Build history of the part. All positions in model axes, mm. A direction names the side the tool comes from. Round coordinates to 2 decimals unless told otherwise and drop trailing zeros. Write each loop counter-clockwise with the first axis right and the second up, starting at its lowest first coordinate (ties: lowest second). Pieces come first, ordered by that corner, then holes. Notation, with made-up numbers: M 39,36.25 L 56,36.25 A23 ccw 56,68.25 Z; hole C 40.25,6.5 d10. An arc over 180 degrees is marked long. Write item = value, one per line. Start each with the question number.
Q1. Tool access for faces 1 (the cylindrical face through (6.466, -2.681, 433.632)), 2 (the flat face through (2, 6, -376.8)): list every direction of +Z, -Z, +X, -X, +Y, -Y with a clear straight run to the whole face (end or side of a thin tool).
Q2. Band-saw the part on A-A on z = -255. Write the cut outline in (x, y).
Q3. Probe L1, parallel to Y at x = 0, z = -391.5; L2, parallel to X at y = 0, z = -393.25; L3, parallel to Z at x = 0.75, y = -7. List the from-to ranges inside material, lowest first.
Q4. Drop flat-ended pins along their axis: P1, Ø2, axis at y = 6.5, z = -155.5, coming from the -X side; P2, Ø1.5, axis at x = 3.5, y = -6, coming from the -Z side; P3, Ø1.1, axis at y = 5, z = -387, coming from the -X side. Give the stop position or say it passes through.
```python
from build123d import *

# Parameters (mm, degrees)
SKETCH_1_R               = 7
EXTRUDE_1_DEPTH          = 450
SKETCH_2_R               = 8.5
EXTRUDE_2_DEPTH          = 416.8
CUT_EXTRUDE_START        = -33.2
SKETCH_3_R               = 8.5
SKETCH_3_R_2             = 6
CUT_EXTRUDE_1_DEPTH      = 33.2
CUT_EXTRUDE_2_DEPTH      = 451.160526923
CUT_EXTRUDE_2_DEPTH_BACK = 451.160526923
SKETCH_4_W               = 12
SKETCH_4_H               = 12.45
MOVE_FACE_1_BY           = 40
MOVE_FACE_1_2_BY         = 40
CUT_EXTRUDE_11_DEPTH     = 2.5
HOLE_WIZARD_M4_1_D       = 3.3
HOLE_WIZARD_M4_1_DEPTH   = 10.1
HOLE_WIZARD_M4_1_TIP     = 0.991420021
CUT_EXTRUDE_START_2      = 1.1
SKETCH_35_R              = 8.5
SKETCH_35_R_2            = 8.1
CUT_EXTRUDE_12_DEPTH     = 1.1
SKETCH_36_R              = 8.5
SKETCH_36_R_2            = 8.1
CUT_EXTRUDE_13_DEPTH     = 1.1
SKETCH_37_R              = 8.5
SKETCH_37_R_2            = 8.1
CUT_EXTRUDE_14_DEPTH     = 1.1
SKETCH_38_R              = 8.5
SKETCH_38_R_2            = 8.1
CUT_EXTRUDE_15_DEPTH     = 1.1


with BuildPart() as part:
    # 草图1 → 凸台-拉伸1 (new, symmetric)
    with BuildSketch(Plane.XY):
        Circle(SKETCH_1_R)
    extrude(amount=EXTRUDE_1_DEPTH, both=True)

    # 草图2 → 凸台-拉伸2 (add, symmetric)
    with BuildSketch(Plane.XY):
        Circle(SKETCH_2_R)
    extrude(amount=EXTRUDE_2_DEPTH, both=True)

    # 草图3 → 切除-拉伸1 (cut)
    with BuildSketch(Plane(origin=(0, 0, -450), x_dir=(-1, 0, 0), z_dir=(0, 0, -1)).offset(CUT_EXTRUDE_START)):
        with Locations(Location((0, 0, 0), (0, 0, 180))):
            Circle(SKETCH_3_R)
        Circle(SKETCH_3_R_2, mode=Mode.SUBTRACT)
    extrude(amount=CUT_EXTRUDE_1_DEPTH, mode=Mode.SUBTRACT)

    # 草图4 → 切除-拉伸2 (cut, two sides: drawn at the far end of the back side and taken through both)
    with BuildSketch(Plane(origin=(0, 0, 0), x_dir=(1, 0, 0), z_dir=(0, 1, 0)).offset(-CUT_EXTRUDE_2_DEPTH_BACK)):
        with Locations((0, 443.775)):
            Rectangle(SKETCH_4_W, SKETCH_4_H)
    extrude(amount=CUT_EXTRUDE_2_DEPTH + CUT_EXTRUDE_2_DEPTH_BACK, mode=Mode.SUBTRACT)

    # Move Face 1: a face moved inward by 40.0
    extrude(part.faces().sort_by_distance((0, 0, -437.55))[0], amount=MOVE_FACE_1_BY, dir=(0, 0, 1), mode=Mode.SUBTRACT)

    # Move Face 1 2: a face moved inward by 40.0
    extrude(part.faces().sort_by_distance((0, -6.8, -416.8))[0], amount=MOVE_FACE_1_2_BY, dir=(0, 0, 1), mode=Mode.SUBTRACT)

    # 草图31 → 切除-拉伸11 (cut)
    with BuildSketch(Plane(origin=(0, 6, -397.55), x_dir=(0, 0, 1), z_dir=(0, 1, 0))):
        with BuildLine():
            Line((-1, 2), (17.75, 2))
            ThreePointArc((17.75, 2), (19.75, 0), (17.75, -2))
            Line((17.75, -2), (-1, -2))
            ThreePointArc((-1, -2), (-3, 0), (-1, 2))
        make_face()
    extrude(amount=-CUT_EXTRUDE_11_DEPTH, mode=Mode.SUBTRACT)

    # M4 螺纹孔1
    with Locations(Plane(origin=(0, 0, -397.55), x_dir=(-1, 0, 0), z_dir=(0, 0, -1))):
        with Locations((0, 0)):
            Hole(HOLE_WIZARD_M4_1_D / 2, depth=HOLE_WIZARD_M4_1_DEPTH)
            with Locations((0, 0, -(HOLE_WIZARD_M4_1_DEPTH + HOLE_WIZARD_M4_1_TIP / 2))):  # 118° drill point
                Cone(0, HOLE_WIZARD_M4_1_D / 2, HOLE_WIZARD_M4_1_TIP, mode=Mode.SUBTRACT)

    # 草图35 → 切除-拉伸12 (cut)
    with BuildSketch(Plane.XY.offset(319.2).offset(CUT_EXTRUDE_START_2)):
        Circle(SKETCH_35_R)
        Circle(SKETCH_35_R_2, mode=Mode.SUBTRACT)
    extrude(amount=-CUT_EXTRUDE_12_DEPTH, mode=Mode.SUBTRACT)

    # 草图36 → 切除-拉伸13 (cut)
    with BuildSketch(Plane.XY.offset(298.1).offset(CUT_EXTRUDE_START_2)):
        Circle(SKETCH_36_R)
        Circle(SKETCH_36_R_2, mode=Mode.SUBTRACT)
    extrude(amount=-CUT_EXTRUDE_13_DEPTH, mode=Mode.SUBTRACT)

    # 草图37 → 切除-拉伸14 (cut)
    with BuildSketch(Plane.XY.offset(-325.8).offset(CUT_EXTRUDE_START_2)):
        Circle(SKETCH_37_R)
        Circle(SKETCH_37_R_2, mode=Mode.SUBTRACT)
    extrude(amount=-CUT_EXTRUDE_14_DEPTH, mode=Mode.SUBTRACT)

    # 草图38 → 切除-拉伸15 (cut)
    with BuildSketch(Plane.XY.offset(-346.9).offset(CUT_EXTRUDE_START_2)):
        Circle(SKETCH_38_R)
        Circle(SKETCH_38_R_2, mode=Mode.SUBTRACT)
    extrude(amount=-CUT_EXTRUDE_15_DEPTH, mode=Mode.SUBTRACT)


solid = part.part
```
Conclusion:
q1.face_1 = +Z
q1.face_2 = -Z
q2.outline = C 0,0 d17
q3.L1 = -6 to -1.65, 1.65 to 3.5
q3.L2 = -6 to -1.65, 1.65 to 6
q3.L3 = -376.8 to 416.8
q4.P1 = -6.48
q4.P2 = -376.8
q4.P3 = -4.02
